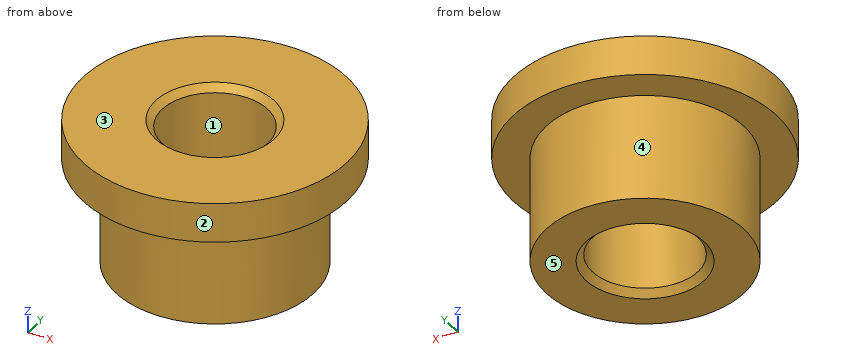
from build123d import *

# Parameters (mm, degrees)
SKETCH_1_R      = 7.5
SKETCH_1_R_2    = 4
EXTRUDE_1_DEPTH = 8
EXTRUDE_START   = 3
SKETCH_2_R      = 10
SKETCH_2_R_2    = 4
EXTRUDE_2_DEPTH = 3
CHAMFER_1_SIZE  = 0.5


with BuildPart() as part:
    # 草图1 → 凸台-拉伸1 (new body)
    with BuildSketch(Plane.XY):
        with Locations((145.504664302, 180.568940096)):
            Circle(SKETCH_1_R)
        with Locations((145.504664302, 180.568940096)):
            Circle(SKETCH_1_R_2, mode=Mode.SUBTRACT)
    extrude(amount=-EXTRUDE_1_DEPTH)

    # 草图2 → 凸台-拉伸2 (add)
    with BuildSketch(Plane.XY.offset(EXTRUDE_START)):
        with Locations((145.504664302, 180.568940096)):
            Circle(SKETCH_2_R)
        with Locations((145.504664302, 180.568940096)):
            Circle(SKETCH_2_R_2, mode=Mode.SUBTRACT)
    extrude(amount=-EXTRUDE_2_DEPTH)

    # 倒角1
    chamfer_1_edges = [part.edges().sort_by_distance(p)[0] for p in [
        (141.504664302, 180.568940096, 3),
        (141.504664302, 180.568940096, -8),
    ]]
    chamfer(chamfer_1_edges, length=CHAMFER_1_SIZE)


solid = part.part
Build history of the part. All positions in model axes, mm. Face numbers are marked on the shaded views. A direction names the side the tool comes from. Give positions to 0.01 mm unless a question says otherwise; leave off trailing zeros. Loops run counter-clockwise (first coordinate to the right, second up) from the corner with the lowest first, then second, coordinate; pieces in that order, holes last. Notation, with made-up numbers: (10, -11) - (24, -11) arc R10 ccw to (24, -5) - close; hole circle Ø11 at (60, 74). An arc over 180 degrees is marked (long way). Write item = value, one per line. Start each with the question number.
1) Probe probe 1 along Y at (x, z) = (145.25, -4.5); probe 2 along X at (y, z) = (180, -6.25); probe 3 along Y at (x, z) = (151.5, -3.25). List the from-to ranges inside material, lowest first. Write a range as from..to.
2) Band-saw the part on A-A on x = 139.5. Give the cut face in (y, z), plus the area to 3 significant figures.
3) Band-saw the part on B-B on y = 174.5. Give the cut face in (x, z).
4) Tool access for the marked faces 4 and 5: list every direction of +Z, -Z, +X, -X, +Y, -Y with a clear straight run to the whole face (end or side of a thin tool).
5) Drop flat-ended pins along their axis: pin 1 Ø3 at (x, z) = (150, -6.5) entering from +Y; pin 2 Ø3 at (x, z) = (138, -2) entering from +Y; pin 3 Ø6 at (y, z) = (174.5, 1) entering from -X. Give the stop position or say it passes through.
6) Pull direction X, two halves, no side cores. Call the marked faces 1, 2 and 3: +X half, -X half, draft (parallel to the pull), parting line (faces both ways), or undercut.
7) Band-saw the part on D-D on z = -4.5. Give the cut face in (x, y).
8) Band-saw the part on C-C on z = 1.25. Give the cut face in (x, y), plus the area to 3 significant figures.
Final values:
q1.probe_1 = 173.07..176.58, 184.56..188.06
q1.probe_2 = 138.03..141.55, 149.46..152.98
q1.probe_3 = 176.06..185.08
q2.outline = (172.57, 0) - (176.08, 0) - (176.08, -8) - (185.06, -8) - (185.06, 0) - (188.57, 0) - (188.57, 3) - (172.57, 3) - close
q2.area = 120 mm²
q3.outline = (137.56, 0) - (141.1, 0) - (141.1, -8) - (149.91, -8) - (149.91, 0) - (153.45, 0) - (153.45, 3) - (137.56, 3) - close
q4.face_4 = -Z
q4.face_5 = -Z, +X, -X, +Y, -Y
q5.pin_1 = 187.44
q5.pin_2 = 185.06
q5.pin_3 = 135.99
q6.face_1 = undercut
q6.face_2 = parting line
q6.face_3 = draft
q7.outline = circle Ø15 at (145.5, 180.57); hole circle Ø8 at (145.5, 180.57)
q8.outline = circle Ø20 at (145.5, 180.57); hole circle Ø8 at (145.5, 180.57)
q8.area = 264 mm²
